```python
from build123d import *

# Parameters (mm, degrees)
EXTRUDE_THIN1_DEPTH = 75
SKETCH2_R           = 25.5
CUT_EXTRUDE1_DEPTH  = 140.143810498
SKETCH4_R           = 3.5
CUT_EXTRUDE3_DEPTH  = 132.335448376
M4_TAPPED_HOLE1_D   = 3.3


with BuildPart() as part:
    # Sketch1 → Extrude-Thin1 (new body)
    with BuildSketch(Plane.XY):
        Polygon((-70, 0), (-50, 0), (-50, 82), (50, 82), (50, 0), (70, 0), (70, -12), (38, -12), (38, 70), (-38, 70), (-38, -12), (-70, -12), align=None)
    extrude(amount=EXTRUDE_THIN1_DEPTH)

    # Sketch2 → Cut-Extrude1 (cut, through all)
    with BuildSketch(Plane(origin=(0, 82, 0), x_dir=(1, 0, 0), z_dir=(0, 1, 0))):
        with Locations(Location((0, -42.5, 0), (0, 0, 270))):
            Circle(SKETCH2_R)
    extrude(amount=-CUT_EXTRUDE1_DEPTH, mode=Mode.SUBTRACT)

    # Sketch4 → Cut-Extrude3 (cut, through all)
    with BuildSketch(Plane(origin=(0, 0, 0), x_dir=(1, 0, 0), z_dir=(0, 1, 0))):
        with Locations(Location((-58, -15, 0), (0, 0, 270))):
            Circle(SKETCH4_R)
        with Locations(Location((58, -15, 0), (0, 0, 90))):
            Circle(SKETCH4_R)
        with Locations(Location((58, -55, 0), (0, 0, 270))):
            Circle(SKETCH4_R)
        with Locations(Location((-58, -55, 0), (0, 0, 90))):
            Circle(SKETCH4_R)
    extrude(amount=-CUT_EXTRUDE3_DEPTH, mode=Mode.SUBTRACT)

    # M4 Tapped Hole1 (through all)
    with Locations(Plane(origin=(0, 82, 0), x_dir=(1, 0, 0), z_dir=(0, 1, 0))):
        with Locations((-24.748737342, -17.751262658), (24.748737342, -17.751262658), (24.748737342, -67.248737342), (-24.748737342, -67.248737342)):
            Hole(M4_TAPPED_HOLE1_D / 2)


solid = part.part
```
Can you work these out from the model? Positions are in its coordinate system, mm. A direction names the side the tool comes from. Coordinates: 2 decimals unless noted, no trailing zeros. Order: outer loops, then holes, each group sorted by start corner. A loop starts at its lowest first (then second) coordinate and runs counter-clockwise, first axis right, second up.
1. For faces 1 (the face through (38, 28, 37)), 2 (the face through (70, -6, 37)), 3 (the face through (-60, 0, 37)), 4 (the face through (50, 42, 37)), which set-ups out of +Z, -Z, +X, -X, +Y, -Y let a thin tool reach every point of the face, with its end or its side?
2. If we section it at B-B (y = 33): Please give me the cut outline in (x, z), then the cut area to 3 significant figures.
3. I'm going to push flat-ended pins straight in: pin 1 (1.5 mm diameter, centred on y = 34.5, z = 37.5, fed in from +X); pin 2 (8 mm diameter, centred on x = -58, z = 15, fed in from -Y); pin 3 (6 mm diameter, centred on y = 34.5, z = 22.5, fed in from -X); pin 4 (5.5 mm diameter, centred on x = -24.75, z = 67.25, fed in from -Y). Where does each tip first touch, or does it pass through?
4. I need wall thicknesses on line 1 (X direction, y = 15.5, z = 55.5); line 2 (X direction, y = -5.5, z = 55); line 3 (X direction, y = 78, z = 42.5). Which ranges of each line are inside material? Lowest first, please.
5. If we section it at D-D (z = 21): Please give me the cut outline in (x, y).
6. If we section it at A-A (x = 58): Please give me the cut outline in (y, z).
7. If we section it at C-C (x = 0): Please give me the cut outline in (y, z).
8. Thinking about a two-plate mould opening in Z: for faces 5 (the face through (11, 74, 75)), 6 (the face through (60, 0, 37)), 7 (the face through (-24.39, 75.92, 19.36)), which applies, +Z half, -Z half, draft (parallel to the pull), parting line (faces both ways), or undercut?
Entries:
1. face 1: +Z, -Z, -Y
1. face 2: +Z, -Z, +X, +Y, -Y
1. face 3: +Z, -Z, -X, +Y
1. face 4: +Z, -Z, +X, +Y
2. outline: (-50, 0) - (-38, 0) - (-38, 75) - (-50, 75) - close; (38, 0) - (50, 0) - (50, 75) - (38, 75) - close
2. area: 1,800 mm2
3. pin 1: stops at x = 50
3. pin 2: stops at y = -12
3. pin 3: stops at x = -50
3. pin 4: stops at y = 70
4. line 1: x = -50 to -38, 38 to 50
4. line 2: x = -70 to -61.5, -54.5 to -38, 38 to 54.5, 61.5 to 70
4. line 3: x = -50 to -25.5, 25.5 to 50
5. outline: (-70, -12) - (-38, -12) - (-38, 70) - (-13.71, 70) - (-13.71, 82) - (-50, 82) - (-50, 0) - (-70, 0) - close; (13.71, 70) - (38, 70) - (38, -12) - (70, -12) - (70, 0) - (50, 0) - (50, 82) - (13.71, 82) - close
6. outline: (-12, 0) - (0, 0) - (0, 11.5) - (-12, 11.5) - close; (-12, 18.5) - (0, 18.5) - (0, 51.5) - (-12, 51.5) - close; (-12, 58.5) - (0, 58.5) - (0, 75) - (-12, 75) - close
7. outline: (70, 0) - (82, 0) - (82, 17) - (70, 17) - close; (70, 68) - (82, 68) - (82, 75) - (70, 75) - close
8. face 5: +Z half
8. face 6: draft
8. face 7: undercut
